Could you check a few things on this drawing? It's one solid part, dimensions in mm from its lowest x, y, z. A direction names the side the tool comes from. Coordinates: 2 decimals unless noted, no trailing zeros. Order: outer loops, then holes, each group sorted by start corner. A loop starts at its lowest first (then second) coordinate and runs counter-clockwise, first axis right, second up. Notation, with made-up numbers: (85, 4) - (107, 4) arc R38 ccw to (107, 42) - close; hole circle Ø2 at (43, 17). An arc over 180 degrees is marked (long way). Return JSON: item names as keys, results as strings. Group by question number.
1) Imagine slicing it at C-C (y = 6.25). Write out the boundary of the cut face in (x, z).
2) Imagine slicing it at D-D (y = 9). Write out the boundary of the cut face in (x, z), and give its area (3 significant figures).
3) Imagine slicing it at A-A (z = 20). Write out the boundary of the cut face in (x, y), and give its area (3 significant figures).
4) Which directions (+Z, -Z, +X, -X, +Y, -Y) give clear straight access to the entire face, cutting with the end or side of a thin tool? Please do the marked faces 1 and 2.
5) If I drill on line 1 along Z through (x, y) = (2.35, 5.75); line 2 along Z through (x, y) = (4.65, 2.75); line 3 along Y through (x, z) = (0.65, 5), over which ranges is the centre line in solid material (lowest first)?
6) If we mould it in two halves opening along Z, with no side actions, what happens to the marked faces 3, 4 and 5? For each: pulls with the +Z half, pulls with the -Z half, needs draft (parallel to the pull), parting line crosses it, or undercut.
7) Imagine slicing it at B-B (x = 3.9). Write out the boundary of the cut face in (y, z), and give its area (3 significant figures).
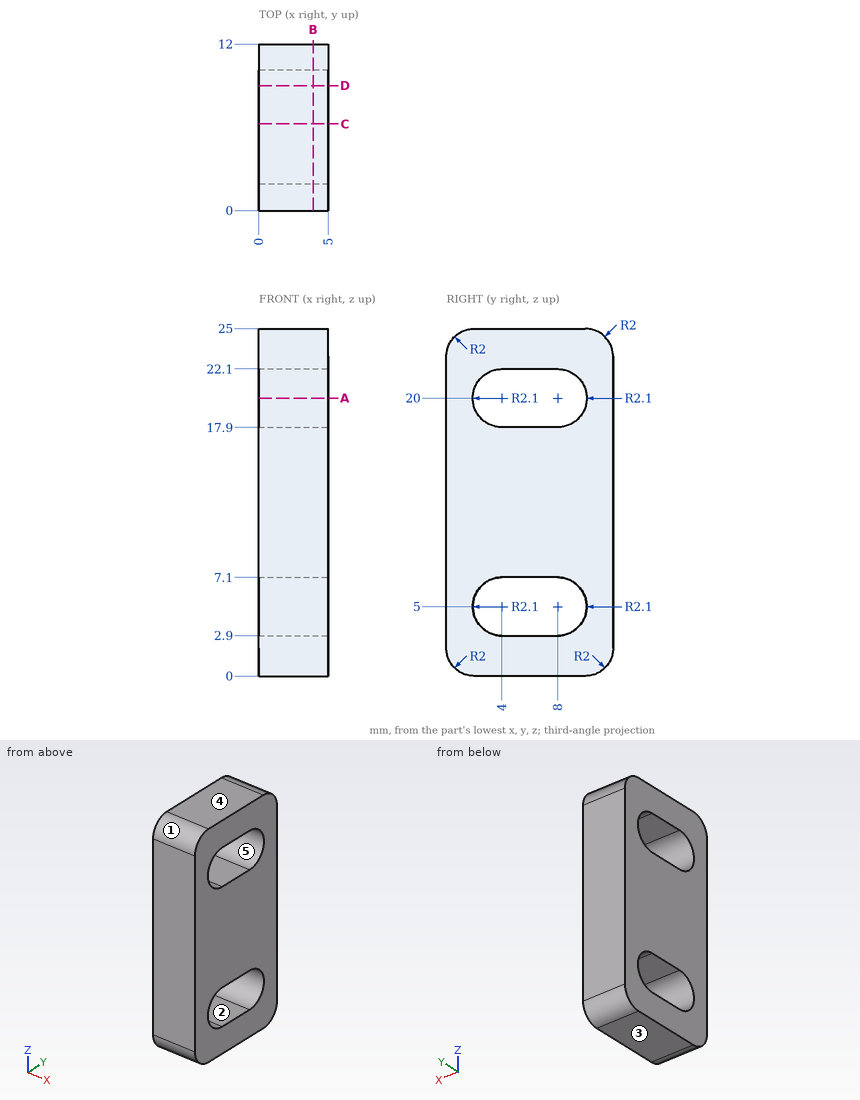
Calculated:
{
 "1": {"outline": "(0, 0) - (5, 0) - (5, 2.9) - (0, 2.9) - close; (0, 7.1) - (5, 7.1) - (5, 17.9) - (0, 17.9) - close; (0, 22.1) - (5, 22.1) - (5, 25) - (0, 25) - close"},
 "2": {"outline": "(0, 0) - (5, 0) - (5, 3.15) - (0, 3.15) - close; (0, 6.85) - (5, 6.85) - (5, 18.15) - (0, 18.15) - close; (0, 21.85) - (5, 21.85) - (5, 25) - (0, 25) - close", "area": "88.1 mm2"},
 "3": {"outline": "(0, 0) - (5, 0) - (5, 1.9) - (0, 1.9) - close; (0, 10.1) - (5, 10.1) - (5, 12) - (0, 12) - close", "area": "19.0 mm2"},
 "4": {"face 1": "+Z, +X, -X, -Y", "face 2": "+X, -X"},
 "5": {"line 1": "0 to 2.9, 7.1 to 17.9, 22.1 to 25", "line 2": "0 to 3.31, 6.69 to 18.31, 21.69 to 25", "line 3": "0 to 1.9, 10.1 to 12"},
 "6": {"face 3": "pulls with the -Z half", "face 4": "pulls with the +Z half", "face 5": "undercut"},
 "7": {"outline": "(0, 2) arc R2 ccw to (2, 0) - (10, 0) arc R2 ccw to (12, 2) - (12, 23) arc R2 ccw to (10, 25) - (2, 25) arc R2 ccw to (0, 23) - close; hole (4, 2.9) - (8, 2.9) arc R2.1 ccw to (8, 7.1) - (4, 7.1) arc R2.1 ccw to start; hole (4, 17.9) - (8, 17.9) arc R2.1 ccw to (8, 22.1) - (4, 22.1) arc R2.1 ccw to start", "area": "235 mm2"}
}
